from build123d import *

# Parameters (mm, degrees)
EXTRUDE_1_DEPTH          = 15
CUT_EXTRUDE_1_DEPTH      = 84.464378629
CUT_EXTRUDE_1_DEPTH_BACK = 84.464378629
SKETCH_2_R               = 2.55
SKETCH_2_R_2             = 2.1
FILLET_1_R               = 3


with BuildPart() as part:
    # 草图1 → 凸台-拉伸1 (new body)
    with BuildSketch(Plane(origin=(0, 0, 0), x_dir=(1, 0, 0), z_dir=(0, 1, 0))):
        Polygon((0, 0), (0, -4), (30.895415868, -4), (41.881332757, -45), (70.55, -45), (70.55, -42), (46.253866082, -42), (35, 0), align=None)
    extrude(amount=EXTRUDE_1_DEPTH)

    # 草图2 → 切除-拉伸1 (cut, two sides: drawn at the far end of the back side and taken through both)
    with BuildSketch(Plane(origin=(0, 0, 42), x_dir=(-1, 0, 0), z_dir=(0, 0, -1)).offset(-CUT_EXTRUDE_1_DEPTH_BACK)):
        with Locations((-63.05, 7.5)):
            Circle(SKETCH_2_R)
        with Locations((-25, 7.5)):
            Circle(SKETCH_2_R_2)
        with Locations((-5, 7.5)):
            Circle(SKETCH_2_R_2)
    extrude(amount=CUT_EXTRUDE_1_DEPTH + CUT_EXTRUDE_1_DEPTH_BACK, mode=Mode.SUBTRACT)

    # 圆角1
    fillet_1_edges = [part.edges().sort_by_distance(p)[0] for p in [
        (35, 7.5, 0),
        (46.253866082, 7.5, 42),
        (41.881332757, 7.5, 45),
        (30.895415868, 7.5, 4),
    ]]
    fillet(fillet_1_edges, radius=FILLET_1_R)


solid = part.part
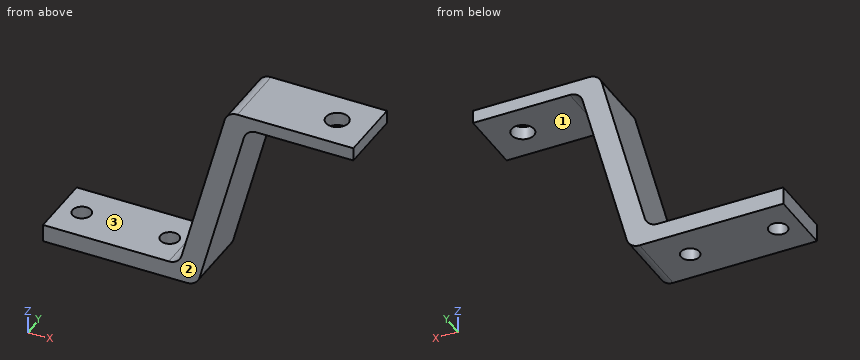
For this review, take the finished solid that the model builds, in its own axes (mm). Face numbers are marked on the shaded views. A direction names the side the tool comes from. Coordinates: 2 decimals unless noted, no trailing zeros. Loops run counter-clockwise (first coordinate to the right, second up) from the corner with the lowest first, then second, coordinate; pieces in that order, holes last. Notation, with made-up numbers: (11.5, 50) - (59.5, 50) arc R21 cw to (59.5, 88) - close; hole circle Ø11 at (-16, 85.5). An arc over 180 degrees is marked (long way). Use a Markdown table: item, result. Add a question column.
Item 1: For line 1 (X direction, y = 7.5, z = 2.75); line 2 (X direction, y = 7.5, z = 1.6); line 3 (Y direction, x = 25, z = 1.3), list the stretches that pass through material, from the lowest coordinate up.
Item 2: Tool access review of the marked faces 1, 2 and 3: name each direction out of +Z, -Z, +X, -X, +Y, -Y from which nothing blocks a thin tool from reaching the whole face with its end or side.
Item 3: Insertion check: pin 1 Ø2.5 at (x, y) = (25, 7.5) entering from -Z (3 decimals); pin 2 Ø1 at (x, y) = (7.5, 3.5) entering from -Z; pin 3 Ø6 at (y, z) = (3, 35.5) entering from +X; pin 4 Ø7.5 at (x, y) = (13.5, 10.5) entering from +Z. Each pin has a flat end and moves straight along its axis. Give the tip position at first contact, or say it passes through.
Item 4: We need section C-C (x = 5). Give the boundary of the cut face in (y, z).
Item 5: We need section D-D (z = 40.5). Give the boundary of the cut face in (x, y).
Item 6: We need section A-A (x = 63.05). Give the boundary of the cut face in (y, z), and give its area (3 significant figures).
Item 7: We need section B-B (y = 7.5). Give the boundary of the cut face in (x, z).
Results list:
| question | item | result |
|---|---|---|
| 1 | line 1 | x = 0 to 2.9, 7.1 to 22.9, 27.1 to 35.74 |
| 1 | line 2 | x = 0 to 2.9, 7.1 to 22.9, 27.1 to 35.35 |
| 1 | line 3 | y = 0 to 5.4, 9.6 to 15 |
| 2 | face 1 | -Z, +X, +Y, -Y |
| 2 | face 2 | +Z, -Z, +X, -X, -Y |
| 2 | face 3 | +Z, -X, +Y, -Y |
| 3 | pin 1 | passes through |
| 3 | pin 2 | stops at z = 0 |
| 3 | pin 3 | stops at x = 45.32 |
| 3 | pin 4 | stops at z = 4 |
| 4 | outline | (0, 0) - (5.4, 0) - (5.4, 4) - (0, 4) - close; (9.6, 0) - (15, 0) - (15, 4) - (9.6, 4) - close |
| 5 | outline | (40.68, 0) - (45.96, 0) - (45.96, 15) - (40.68, 15) - close |
| 6 | outline | (0, 42) - (4.95, 42) - (4.95, 45) - (0, 45) - close; (10.05, 42) - (15, 42) - (15, 45) - (10.05, 45) - close |
| 6 | area | 29.7 mm^2 |
| 7 | outline | (0, 0) - (2.9, 0) - (2.9, 4) - (0, 4) - close; (7.1, 0) - (22.9, 0) - (22.9, 4) - (7.1, 4) - close; (27.1, 0) - (32.7, 0) arc R3 ccw to (35.6, 2.22) - (45.66, 39.78) arc R3 cw to (48.56, 42) - (60.5, 42) - (60.5, 45) - (44.18, 45) arc R3 ccw to (41.29, 42.78) - (31.49, 6.22) arc R3 cw to (28.59, 4) - (27.1, 4) - close; (65.6, 42) - (70.55, 42) - (70.55, 45) - (65.6, 45) - close |
